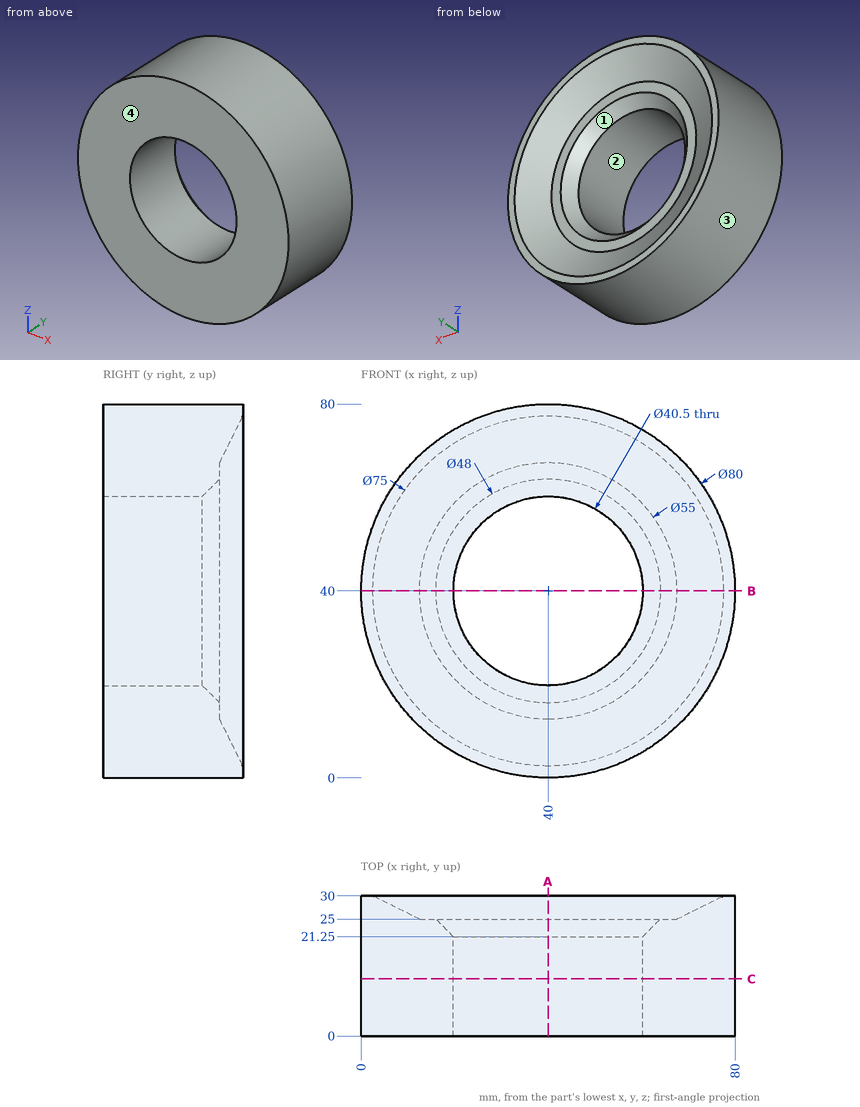
Geometry check sheet. Reference: drawing and pictorial views, mm from the part's lowest x, y, z. Give positions to 0.01 mm unless a question says otherwise; leave off trailing zeros. Write each loop counter-clockwise with the first axis right and the second up, starting at its lowest first coordinate (ties: lowest second). Pieces come first, ordered by that corner, then holes.
Item 1: Gauge pin test, flat ends, axial feed: pin 1 (5 mm diameter, centred on y = 24, z = 53.5, fed in from +X); pin 2 (1.5 mm diameter, centred on y = 8.5, z = 56.5, fed in from -X); pin 3 (2 mm diameter, centred on x = 32, y = 8, fed in from +Z). Record the tip position at first contact, or that the pin passes through.
Item 2: Cross-section at B-B (z = 40). Enter the section's corners in (x, y).
Item 3: Draft check along Z on the marked faces 1, 2, 3 and 4. Enter one of: released by +Z, released by -Z, zero draft, split by the parting line, or undercut.
Item 4: Cross-section at A-A (x = 40). Enter the section's corners in (y, z), and give its area (3 significant figures).
Item 5: Scan lines: L1, parallel to Z at x = 8, y = 18.5; L2, parallel to X at y = 24.5, z = 38.5; L3, parallel to Z at x = 22.5, y = 11.25. Record each from-to range of solid material in increasing order.
Item 6: Cross-section at C-C (y = 12.25). Enter the section's corners in (x, z), and give its area (3 significant figures).
Report:
1. pin 1: stops at x = 78.46
1. pin 2: stops at x = 3.23
1. pin 3: stops at z = 79.38
2. outline: (0, 0) - (19.75, 0) - (19.75, 21.25) - (16, 25) - (12.5, 25) - (2.5, 30) - (0, 30) - close; (60.25, 0) - (80, 0) - (80, 30) - (77.5, 30) - (67.5, 25) - (64, 25) - (60.25, 21.25) - close
3. face 1: undercut
3. face 2: undercut
3. face 3: split by the parting line
3. face 4: zero draft
4. outline: (0, 0) - (30, 0) - (30, 2.5) - (25, 12.5) - (25, 16) - (21.25, 19.75) - (0, 19.75) - close; (0, 60.25) - (21.25, 60.25) - (25, 64) - (25, 67.5) - (30, 77.5) - (30, 80) - (0, 80) - close
4. area: 1,050 mm2
5. L1: z = 16 to 64
5. L2: x = 0.03 to 16.55, 63.45 to 79.97
5. L3: z = 4.03 to 29.81, 50.19 to 75.97
6. outline: circle Ø80 at (40, 40); hole circle Ø40.5 at (40, 40)
6. area: 3,740 mm2
